The figure shows three views and two pictorial views of one solid part (mm, origin at its lowest corner). Answer the questions. A direction names the side the tool comes from. Give positions to 0.01 mm unless a question says otherwise; leave off trailing zeros. Write each loop counter-clockwise with the first axis right and the second up, starting at its lowest first coordinate (ties: lowest second). Pieces come first, ordered by that corner, then holes. Notation, with made-up numbers: (-3.5, 1.5) -> (50.5, 1.5) arc R14 cw to (50.5, 16.5) -> close; hole circle Ø6 at (34, -2). An arc over 180 degrees is marked (long way). Use a Markdown table: item, result.
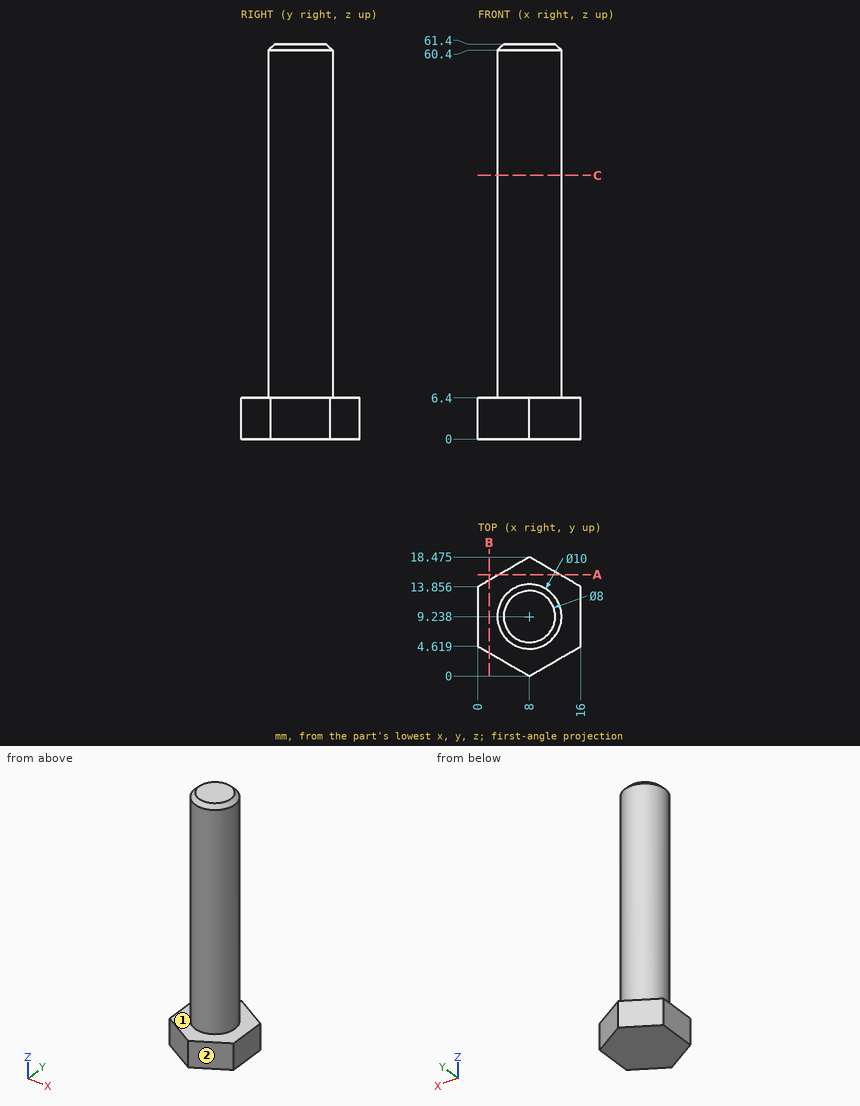
Item 1: A cutting plane is placed at B-B (x = 1.75). Give the vertices of the cut face in (y, z).
Return value:
| item | result |
|---|---|
| outline | (3.61, 0) -> (14.87, 0) -> (14.87, 6.4) -> (3.61, 6.4) -> close |
Item 2: A cutting plane is placed at C-C (z = 41). Give the vertices of the cut face in (x, y).
Return value:
| item | result |
|---|---|
| outline | circle Ø10 at (8, 9.24) |
Item 3: Each of these flat-tipped pins is pushed along its axis until it touches: P1, Ø2, axis at x = 4.5, y = 4, coming from the +Z side; P2, Ø6, axis at x = 11, z = 35, coming from the +Y side; P3, Ø5, axis at y = 4, z = 11, coming from the +X side (1 decimal). Where does it stop, or does it pass through?
Return value:
| item | result |
|---|---|
| P1 | z = 6.4 |
| P2 | y = 14.24 |
| P3 | x = 12.2 |
Item 4: A tool of negligible diameter and unlimited length cuts with its end or side. For the marked faces 1 and 2, from which of +Z, -Z, +X, -X, +Y, -Y can it reach the whole face along a straight path? Write none if from no direction.
Return value:
| item | result |
|---|---|
| face 1 | +Z |
| face 2 | +Z, -Z, +X, -Y |
Item 5: Straight lines are drawn through the part: line 1 along Z through (x, y) = (12.5, 14); line 2 along X through (y, z) = (12.25, 22.5); line 3 along Y through (x, z) = (5.25, 41) (1 decimal). For each, find the intervals that lie inside material, in ascending order. Write a range as [from, to].
Return value:
| item | result |
|---|---|
| line 1 | [0, 6.4] |
| line 2 | [4.01, 11.99] |
| line 3 | [5.1, 13.4] |
Item 6: A cutting plane is placed at A-A (y = 15.75). Give the vertices of the cut face in (x, z), then the cut area to 3 significant figures.
Return value:
| item | result |
|---|---|
| outline | (3.28, 0) -> (12.72, 0) -> (12.72, 6.4) -> (3.28, 6.4) -> close |
| area | 60.4 mm^2 |
